from build123d import *

# Parameters (mm, degrees)
BOSS_EXTRUDE1_DEPTH = 20


with BuildPart() as part:
    # Sketch1 → Boss-Extrude1 (new body)
    with BuildSketch(Plane.XY):
        with BuildLine():
            Line((-124.5, 0), (124.5, 0))
            Line((124.5, 0), (136.5, 12))
            Line((136.5, 12), (136.5, 160.6))
            ThreePointArc((136.5, 160.6), (131.600675284, 175.464819311), (118.822971749, 184.503432489))
            Line((118.822971749, 184.503432489), (10.252160448, 217.764805485))
            ThreePointArc((10.252160448, 217.764805485), (0, 219.3), (-10.252160448, 217.764805485))
            Line((-10.252160448, 217.764805485), (-118.822971749, 184.503432489))
            ThreePointArc((-118.822971749, 184.503432489), (-131.600675284, 175.464819311), (-136.5, 160.6))
            Line((-136.5, 160.6), (-136.5, 12))
            Line((-136.5, 12), (-124.5, 0))
        make_face()
        with BuildLine():
            Line((-21, 123), (21, 123))
            ThreePointArc((21, 123), (31.242640687, 127.242640687), (27, 117))
            Line((27, 117), (27, 75))
            ThreePointArc((27, 75), (31.242640687, 64.757359313), (21, 69))
            Line((21, 69), (-21, 69))
            ThreePointArc((-21, 69), (-31.242640687, 64.757359313), (-27, 75))
            Line((-27, 75), (-27, 117))
            ThreePointArc((-27, 117), (-31.242640687, 127.242640687), (-21, 123))
        make_face(mode=Mode.SUBTRACT)
    extrude(amount=BOSS_EXTRUDE1_DEPTH)


solid = part.part
Input: part model. Units: mm. Frame: model coordinates. A direction names the side the tool comes from. Give positions to 0.01 mm unless a question says otherwise; leave off trailing zeros. Write each loop counter-clockwise with the first axis right and the second up, starting at its lowest first coordinate (ties: lowest second). Pieces come first, ordered by that corner, then holes.
Q1. Section A-A, the plane z = 8.75. Output: boundary loops of the cut face in (x, y), plus the area to 3 significant figures.
Q2. Section C-C, the plane x = -70. Output: boundary loops of the cut face in (y, z), plus the area to 3 significant figures.
Q3. Set-up query: faces 1 (the face through (27, 96, 10)), 2 (the face through (136.5, 85, 10)). Return all of +Z, -Z, +X, -X, +Y, -Y with unobstructed straight access to the full face (end or side cutting, diameter ignored); none if empty.
Q4. First-contact query: P1, Ø6, axis at x = -49, z = 6, coming from the +Y side. Flat tip, straight axial feed; report the tip coordinate or a pass-through.
Q5. Pull-direction query (X, two-part tool) for faces 3 (the face through (0, 123, 10)), 4 (the face through (-130.6, 6.1, 9.9)), 5 (the face through (131.73, 175.29, 9.86)); classes: pulls with the +X half, pulls with the -X half, needs draft (parallel to the pull), parting line crosses it, or undercut.
Q6. Section B-B, the plane x = 87.5. Output: boundary loops of the cut face in (y, z).
Q7. Material intervals for probe 1 along X at (y, z) = (116, 13.5); probe 2 along X at (y, z) = (128.5, 18); probe 3 along Y at (x, z) = (84, 6), sorted ascending.
Filled in:
1. outline: (-136.5, 12) - (-124.5, 0) - (124.5, 0) - (136.5, 12) - (136.5, 160.6) arc R25 ccw to (118.82, 184.5) - (10.25, 217.76) arc R35 ccw to (-10.25, 217.76) - (-118.82, 184.5) arc R25 ccw to (-136.5, 160.6) - close; hole (-27, 75) arc R6 ccw (long way) to (-21, 69) - (21, 69) arc R6 ccw (long way) to (27, 75) - (27, 117) arc R6 ccw (long way) to (21, 123) - (-21, 123) arc R6 ccw (long way) to (-27, 117) - close
1. area: 51,100 mm2
2. outline: (0, 0) - (199.46, 0) - (199.46, 20) - (0, 20) - close
2. area: 3,990 mm2
3. face 1: +Z, -Z
3. face 2: +Z, -Z, +X, +Y, -Y
4. P1: stops at y = 206.81
5. face 3: undercut
5. face 4: pulls with the -X half
5. face 5: pulls with the +X half
6. outline: (0, 0) - (194.1, 0) - (194.1, 20) - (0, 20) - close
7. probe 1: x = -136.5 to -27, 27 to 136.5
7. probe 2: x = -136.5 to -29.4, -24.6 to 24.6, 29.4 to 136.5
7. probe 3: y = 0 to 195.17
